from build123d import *

# Parameters (mm, degrees)
SKETCH1_R              = 30
BOSS_EXTRUDE1_DEPTH    = 1090
SKETCH2_R              = 10
BOSS_EXTRUDE2_DEPTH    = 13
BOSS_EXTRUDE3_START    = 13
SKETCH3_R              = 10
BOSS_EXTRUDE3_DEPTH    = 13
M12_TAPPED_HOLE1_D     = 10.2
M12_TAPPED_HOLE1_DEPTH = 25.25
M12_TAPPED_HOLE1_TIP   = 3.064389157
M12_TAPPED_HOLE2_D     = 10.2
M12_TAPPED_HOLE2_DEPTH = 25.25
M12_TAPPED_HOLE2_TIP   = 3.064389157


with BuildPart() as part:
    # Sketch1 → Boss-Extrude1 (new body)
    with BuildSketch(Plane.XY):
        Circle(SKETCH1_R)
    extrude(amount=BOSS_EXTRUDE1_DEPTH)

    # Sketch2 → Boss-Extrude2 (add)
    with BuildSketch(Plane.XY.offset(1090)):
        with Locations(Location((0, 0, 0), (0, 0, 180))):
            Circle(SKETCH2_R)
    extrude(amount=BOSS_EXTRUDE2_DEPTH)

    # Sketch3 → Boss-Extrude3 (add)
    with BuildSketch(Plane(origin=(0, 0, 0), x_dir=(-1, 0, 0), z_dir=(0, 0, -1)).offset(BOSS_EXTRUDE3_START)):
        Circle(SKETCH3_R)
    extrude(amount=-BOSS_EXTRUDE3_DEPTH)

    # M12 Tapped Hole1
    with Locations(Plane(origin=(0, 0, -13), x_dir=(-1, 0, 0), z_dir=(0, 0, -1))):
        with Locations((0, 0)):
            Hole(M12_TAPPED_HOLE1_D / 2, depth=M12_TAPPED_HOLE1_DEPTH)
            with Locations((0, 0, -(M12_TAPPED_HOLE1_DEPTH + M12_TAPPED_HOLE1_TIP / 2))):  # 118° drill point
                Cone(0, M12_TAPPED_HOLE1_D / 2, M12_TAPPED_HOLE1_TIP, mode=Mode.SUBTRACT)

    # M12 Tapped Hole2
    with Locations(Plane.XY.offset(1103)):
        with Locations((0, 0)):
            Hole(M12_TAPPED_HOLE2_D / 2, depth=M12_TAPPED_HOLE2_DEPTH)
            with Locations((0, 0, -(M12_TAPPED_HOLE2_DEPTH + M12_TAPPED_HOLE2_TIP / 2))):  # 118° drill point
                Cone(0, M12_TAPPED_HOLE2_D / 2, M12_TAPPED_HOLE2_TIP, mode=Mode.SUBTRACT)


solid = part.part
Work out the finished part from the listing and answer in its coordinate system (mm). A direction names the side the tool comes from. Coordinates: 2 decimals unless noted, no trailing zeros. Write each loop counter-clockwise with the first axis right and the second up, starting at its lowest first coordinate (ties: lowest second). Pieces come first, ordered by that corner, then holes. Notation, with made-up numbers: M 60,-26 L 119,-26 A30 cw 119,6 Z; hole C -16.5,56 d9. An arc over 180 degrees is marked long. Write item = value, one per line.
1. Flat-ended cylindrical pins translate along their axes: pin 1 (3 mm diameter, centred on x = 6.5, z = 950, fed in from +Y); pin 2 (6 mm diameter, centred on x = 0, y = 0, fed in from -Z); pin 3 (5 mm diameter, centred on x = 1.5, z = 944, fed in from +Y). Find the tip coordinate at first contact, or state that the pin passes through.
Solution:
pin_1 = 29.58
pin_2 = 13.51
pin_3 = 30
2. Straight lines are drawn through the part: line 1 (Y direction, x = 0, z = 1096); line 2 (Z direction, x = 18.5, y = -2); line 3 (Y direction, x = 3, z = 320). For each, find the intervals that lie inside material, in ascending order. Write a range as from..to.
Solution:
line_1 = -10..-5.1, 5.1..10
line_2 = 0..1090
line_3 = -29.85..29.85
3. The part is cut by section C-C (y = -21). Determine the outline of the cut face in (x, z), then the cut area to 3 significant figures.
Solution:
outline = M -21.42,0 L 21.42,0 L 21.42,1090 L -21.42,1090 Z
area = 46,700 mm2
4. The part is cut by section A-A (z = 560). Determine the outline of the cut face in (x, y).
Solution:
outline = C 0,0 d60
5. The part is cut by section B-B (y = 19). Determine the outline of the cut face in (x, z), then the cut area to 3 significant figures.
Solution:
outline = M -23.22,0 L 23.22,0 L 23.22,1090 L -23.22,1090 Z
area = 50,600 mm2
6. For faces 1 (the face through (10, 0, 1096)), 2 (the face through (13, 0, 0)), 3 (the face through (2, -5, 1103)), determine the directions among +Z, -Z, +X, -X, +Y, -Y from which every point of the face is accessible in a straight line to the end or side of a thin tool.
Solution:
face_1 = +Z
face_2 = -Z
face_3 = +Z, +X, -X, +Y, -Y
